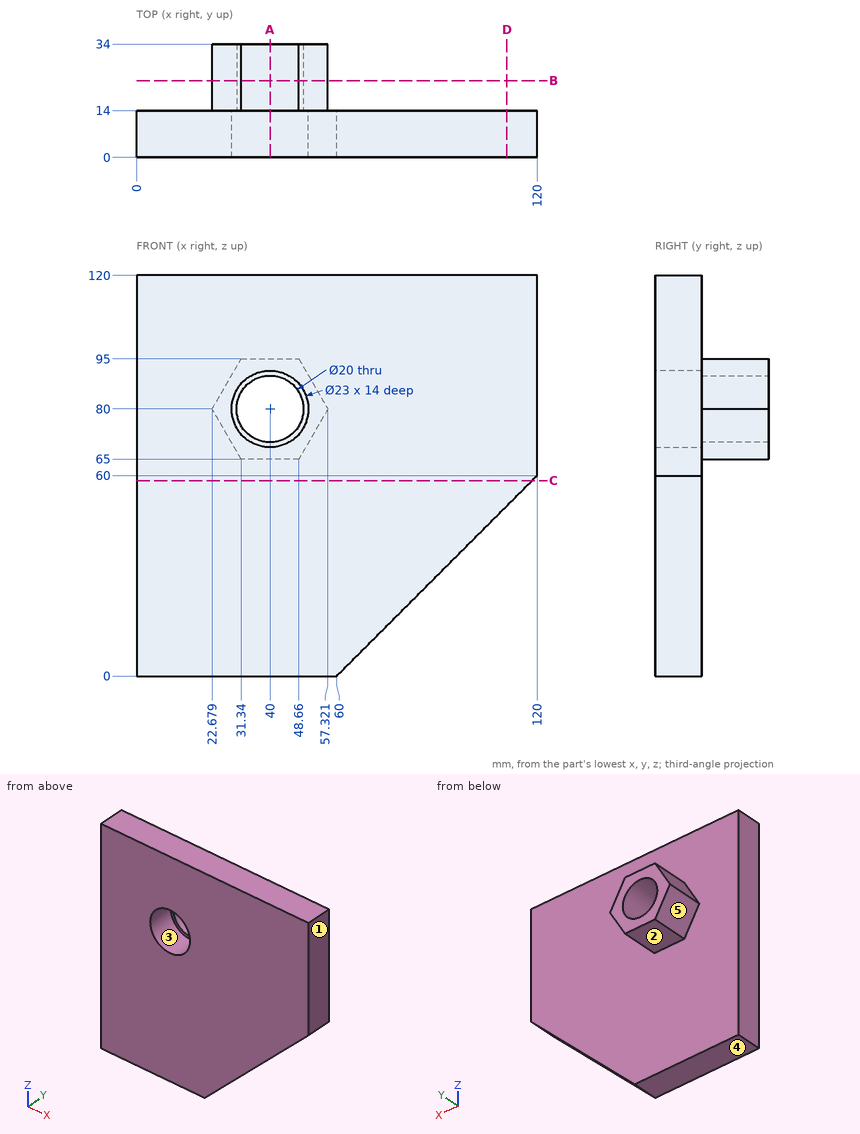
Here's the drawing with two shaded views (mm, measured from the low corner). I have some questions. A direction names the side the tool comes from. Coordinates: 2 decimals unless noted, no trailing zeros. Order: outer loops, then holes, each group sorted by start corner. A loop starts at its lowest first (then second) coordinate and runs counter-clockwise, first axis right, second up. Notation, with made-up numbers: M 45.25,56 L 70.25,56 A24 cw 70.25,89 Z; hole C 83.25,1.5 d1. An arc over 180 degrees is marked long. Write item = value, one per line.
(1) For pin 1 Ø8 at (x, z) = (20.5, 26.5) entering from +Y; pin 2 Ø4 at (x, y) = (61, 26) entering from +Z; pin 3 Ø14 at (x, y) = (36.5, 24) entering from -Z, each with a flat end and sliding along its axis, tell me the tip position at first contact or that it passes through.
Results are:
pin_1 = 14
pin_2 = through
pin_3 = 65
(2) Suppose I cut it at D-D on x = 111. Please give me the cut outline in (y, z).
Results are:
outline = M 0,51 L 14,51 L 14,120 L 0,120 Z
(3) Suppose I cut it at C-C on z = 58.5. Please give me the cut outline in (x, y).
Results are:
outline = M 0,0 L 118.5,0 L 118.5,14 L 0,14 Z
(4) Suppose I cut it at B-B on y = 23. Please give me the cut outline in (x, z).
Results are:
outline = M 22.68,80 L 31.34,65 L 48.66,65 L 57.32,80 L 48.66,95 L 31.34,95 Z; hole C 40,80 d20
(5) For the marked faces 4 and 5, which set-ups out of +Z, -Z, +X, -X, +Y, -Y let a thin tool reach every point of the face, with its end or its side?
Results are:
face_4 = -Z, +X, -X, +Y, -Y
face_5 = -Z, -X, +Y
(6) Suppose I cut it at A-A on x = 40. Please give me the cut outline in (y, z), plus the area to 3 significant figures.
Results are:
outline = M 0,0 L 14,0 L 14,65 L 34,65 L 34,70 L 14,70 L 14,68.5 L 0,68.5 Z; M 0,91.5 L 14,91.5 L 14,90 L 34,90 L 34,95 L 14,95 L 14,120 L 0,120 Z
area = 1,560 mm2
(7) If we mould it in two halves opening along Z, with no side actions, what happens to the marked faces 1, 2 and 3? For each: pulls with the +Z half, pulls with the -Z half, needs draft (parallel to the pull), parting line crosses it, or undercut.
Results are:
face_1 = needs draft
face_2 = pulls with the -Z half
face_3 = undercut
(8) I need wall thicknesses on line 1 along X through (y, z) = (20.75, 80); line 2 along X through (y, z) = (3.75, 80); line 3 along Y through (x, z) = (14, 23). Which ranges of each line are inside material? Lowest first, please. Write a range as [from, to].
Results are:
line_1 = [22.68, 30], [50, 57.32]
line_2 = [0, 28.5], [51.5, 120]
line_3 = [0, 14]
